from build123d import *

# Parameters (mm, degrees)
SKETCH_1_W                   = 60
SKETCH_1_H                   = 120
EXTRUDE_1_DEPTH              = 2
SKETCH_2_W                   = 36
SKETCH_2_H                   = 76
CUT_EXTRUDE_1_DEPTH          = 68.201190466
SKETCH_3_W                   = 40.2
SKETCH_3_H                   = 80.2
CUT_EXTRUDE_2_DEPTH          = 2
HOLE_WIZARD_3_0_3_1_D        = 3
HOLE_WIZARD_3_0_3_1_DEPTH    = 2
FILLET_1_R                   = 3
HOLE_WIZARD_M2_1_D           = 2.4
HOLE_WIZARD_M2_1_CBORE_D     = 4.4
HOLE_WIZARD_M2_1_CBORE_DEPTH = 2.4


with BuildPart() as part:
    # 草图1 → 凸台-拉伸1 (new, symmetric)
    with BuildSketch(Plane.XY):
        Rectangle(SKETCH_1_W, SKETCH_1_H)
    extrude(amount=EXTRUDE_1_DEPTH, both=True)

    # 草图2 → 切除-拉伸1 (cut, through all)
    with BuildSketch(Plane.XY.offset(2)):
        with Locations((-2, 0)):
            Rectangle(SKETCH_2_W, SKETCH_2_H)
    extrude(amount=-CUT_EXTRUDE_1_DEPTH, mode=Mode.SUBTRACT)

    # 草图3 → 切除-拉伸2 (cut)
    with BuildSketch(Plane.XY.offset(2)):
        with Locations((-2, 0)):
            Rectangle(SKETCH_3_W, SKETCH_3_H)
    extrude(amount=-CUT_EXTRUDE_2_DEPTH, mode=Mode.SUBTRACT)

    # Ø3.0 (3) 直径孔1
    with Locations(Plane.XY.offset(2)):
        with Locations((-20.6, 40.1), (16.6, 40.1), (16.6, -40.1), (-20.6, -40.1)):
            Hole(HOLE_WIZARD_3_0_3_1_D / 2, depth=HOLE_WIZARD_3_0_3_1_DEPTH)

    # 圆角1
    fillet_1_edges = [part.edges().sort_by_distance(p)[0] for p in [
        (-20, -38, -1),
        (-20, 38, -1),
        (16, 38, -1),
        (16, -38, -1),
    ]]
    fillet(fillet_1_edges, radius=FILLET_1_R)

    # M2 六角凹头螺钉的柱形沉头孔1 (through all)
    with Locations(Plane(origin=(0, 0, -2), x_dir=(1, 0, 0), z_dir=(0, 0, -1))):
        with Locations((-28, 0), (28, 0), (-15, -58), (15, -58), (-28, -35), (28, -35), (-28, 35), (28, 35), (-15, 58), (15, 58)):
            CounterBoreHole(HOLE_WIZARD_M2_1_D / 2, HOLE_WIZARD_M2_1_CBORE_D / 2, HOLE_WIZARD_M2_1_CBORE_DEPTH)


solid = part.part
The listing builds one solid part. Answer for the finished solid, in the listing's coordinates (mm). A direction names the side the tool comes from. Round coordinates to 2 decimals unless told otherwise and drop trailing zeros. Order: outer loops, then holes, each group sorted by start corner. A loop starts at its lowest first (then second) coordinate and runs counter-clockwise, first axis right, second up. Notation, with made-up numbers: (72.5, 11) - (130.5, 11) arc R15 ccw to (130.5, 37) - close; hole circle Ø4 at (4.5, 15.5). An arc over 180 degrees is marked (long way). Write item = value, one per line. Start each with the question number.
1) Straight lines are drawn through the part: L1, parallel to Y at x = -28, z = 0.9; L2, parallel to Y at x = -28, z = -1.05; L3, parallel to X at y = 35, z = 1.65. For each, find the intervals that lie inside material, in ascending order.
2) For a pull along X with two mould halves and no side action, classify faces 1 (the cylindrical face through (-28.65, 33.99, 1.21)), 2 (the flat face through (-30, -1, 1)), 3 (the flat face through (0, -60, 0)) as released by +X, released by -X, zero draft, split by the parting line, or undercut.
3) Section A-A, the plane y = 58 is taken. Write down the section's boundary in (x, z).
4) Section C-C, the plane y = 17 is taken. Write down the section's boundary in (x, z), plus the area to 3 significant figures.
5) Given pin 1 (3 mm diameter, centred on x = 28, y = -35, fed in from -Z); pin 2 (1.4 mm diameter, centred on x = 28, y = 35, fed in from -Z), each flat-ended and moving along its own axis, determine where each tip first touches the part or whether it passes through.
6) For faces 4 (the flat face through (-29, 36, 0.4)), 5 (the cylindrical face through (15.1, -37.14, -1.01)), 6 (the flat face through (-21, -12, 0)), determine the directions among +Z, -Z, +X, -X, +Y, -Y from which every point of the face is accessible in a straight line to the end or side of a thin tool.
7) Section B-B, the plane x = -28 is taken. Write down the section's boundary in (y, z), plus the area to 3 significant figures.
Results list:
q1.L1 = -60 to -36.2, -33.8 to -1.2, 1.2 to 33.8, 36.2 to 60
q1.L2 = -60 to -37.2, -32.8 to -2.2, 2.2 to 32.8, 37.2 to 60
q1.L3 = -30 to -29.2, -26.8 to -22.1, 18.1 to 26.8, 29.2 to 30
q2.face_1 = undercut
q2.face_2 = released by -X
q2.face_3 = zero draft
q3.outline = (-30, -2) - (-17.2, -2) - (-17.2, 0.4) - (-16.2, 0.4) - (-16.2, 2) - (-30, 2) - close; (-13.8, 0.4) - (-12.8, 0.4) - (-12.8, -2) - (12.8, -2) - (12.8, 0.4) - (13.8, 0.4) - (13.8, 2) - (-13.8, 2) - close; (16.2, 0.4) - (17.2, 0.4) - (17.2, -2) - (30, -2) - (30, 2) - (16.2, 2) - close
q4.outline = (-30, -2) - (-20, -2) - (-20, 0) - (-22.1, 0) - (-22.1, 2) - (-30, 2) - close; (16, -2) - (30, -2) - (30, 2) - (18.1, 2) - (18.1, 0) - (16, 0) - close
q4.area = 87.6 mm^2
q5.pin_1 = 0.4
q5.pin_2 = through
q6.face_4 = -Z
q6.face_5 = +Z, -Z
q6.face_6 = +Z
q7.outline = (-60, -2) - (-37.2, -2) - (-37.2, 0.4) - (-36.2, 0.4) - (-36.2, 2) - (-60, 2) - close; (-33.8, 0.4) - (-32.8, 0.4) - (-32.8, -2) - (-2.2, -2) - (-2.2, 0.4) - (-1.2, 0.4) - (-1.2, 2) - (-33.8, 2) - close; (1.2, 0.4) - (2.2, 0.4) - (2.2, -2) - (32.8, -2) - (32.8, 0.4) - (33.8, 0.4) - (33.8, 2) - (1.2, 2) - close; (36.2, 0.4) - (37.2, 0.4) - (37.2, -2) - (60, -2) - (60, 2) - (36.2, 2) - close
q7.area = 437 mm^2
